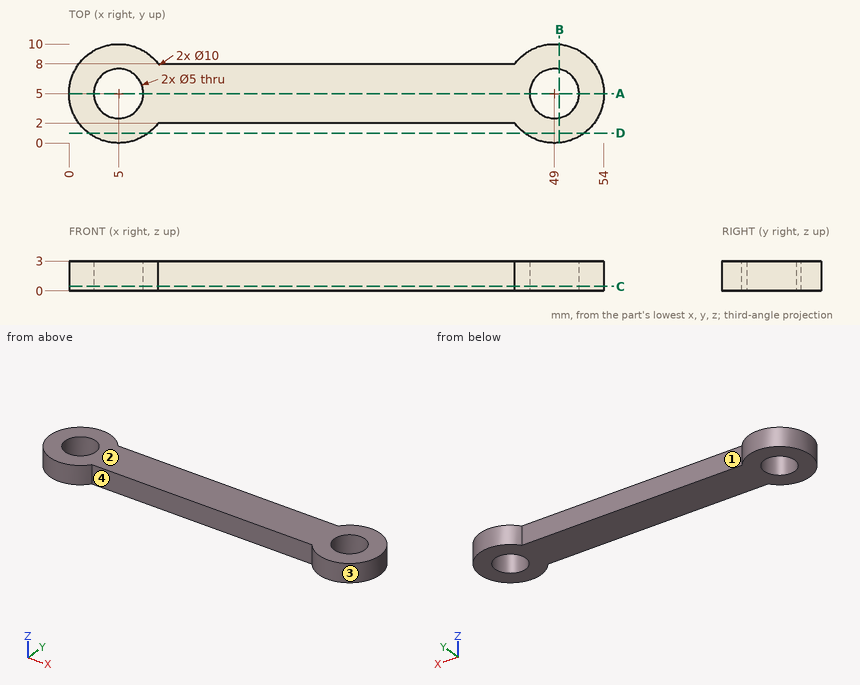
Check sheet for the drawn part. Datum: minimum x, y, z corner. Units: mm. A direction names the side the tool comes from. Round coordinates to 2 decimals unless told otherwise and drop trailing zeros. Loops run counter-clockwise (first coordinate to the right, second up) from the corner with the lowest first, then second, coordinate; pieces in that order, holes last. Notation, with made-up numbers: (-37, -28.5) - (-24, -28.5) arc R7 cw to (-24, -20.5) - close; hole circle Ø5 at (17.25, 32.25). An arc over 180 degrees is marked (long way). Write item = value, one per line. Start each with the question number.
1. Section check A-A on y = 5. Enter the section's corners in (x, z).
2. Set-up check for the marked faces 3 and 4: record each of +Z, -Z, +X, -X, +Y, -Y from which the full face is reachable in a straight line by a thin tool's end or side.
3. Section check B-B on x = 49.5. Enter the section's corners in (y, z).
4. Depth check by flat-ended pin: pin 1 (1.5 mm diameter, centred on x = 32.5, z = 1.5, fed in from +Y); pin 2 (1 mm diameter, centred on y = 6, z = 1.5, fed in from +X); pin 3 (1 mm diameter, centred on x = 33.5, z = 2.5, fed in from -Y); pin 4 (3 mm diameter, centred on x = 5, y = 5, fed in from -Z). Enter the tip coordinate at first touch or a pass-through.
5. Section check C-C on z = 0.45. Enter the section's corners in (x, y), then the cut area to 3 significant figures.
6. Mould release check, pull along X, two halves, no side actions. Record for the marked faces 1 and 2: released by +X, released by -X, zero draft, split by the parting line, or undercut.
7. Section check D-D on y = 1. Enter the section's corners in (x, z), then the cut area to 3 significant figures.
8. Thickness scan on line 1 (Y direction, x = 5, z = 1.4); line 2 (Y direction, x = 10, z = 0.5); line 3 (X direction, y = 4, z = 1.8). Record the ranges inside material, lowest first.
Working result:
q1.outline = (0, 0) - (2.5, 0) - (2.5, 3) - (0, 3) - close; (7.5, 0) - (46.5, 0) - (46.5, 3) - (7.5, 3) - close; (51.5, 0) - (54, 0) - (54, 3) - (51.5, 3) - close
q2.face_3 = +Z, -Z
q2.face_4 = +Z, -Z, -Y
q3.outline = (0.03, 0) - (2.55, 0) - (2.55, 3) - (0.03, 3) - close; (7.45, 0) - (9.97, 0) - (9.97, 3) - (7.45, 3) - close
q4.pin_1 = 8
q4.pin_2 = 53.97
q4.pin_3 = 2
q4.pin_4 = through
q5.outline = (9, 2) - (45, 2) arc R5 ccw (long way) to (45, 8) - (9, 8) arc R5 ccw (long way) to start; hole circle Ø5 at (5, 5); hole circle Ø5 at (49, 5)
q5.area = 326 mm^2
q6.face_1 = undercut
q6.face_2 = zero draft
q7.outline = (2, 0) - (8, 0) - (8, 3) - (2, 3) - close; (46, 0) - (52, 0) - (52, 3) - (46, 3) - close
q7.area = 36.0 mm^2
q8.line_1 = 0 to 2.5, 7.5 to 10
q8.line_2 = 2 to 8
q8.line_3 = 0.1 to 2.71, 7.29 to 46.71, 51.29 to 53.9
